Model file for the job. Use its own axes, mm. Round coordinates to 2 decimals unless told otherwise and drop trailing zeros. Loops run counter-clockwise (first coordinate to the right, second up) from the corner with the lowest first, then second, coordinate; pieces in that order, holes last.
from build123d import *

# Parameters (mm, degrees)
SKETCH_1_W      = 190
SKETCH_1_H      = 50
SKETCH_1_R      = 4.5
EXTRUDE_1_DEPTH = 7.25


with BuildPart() as part:
    # 草图1 → 凸台-拉伸1 (new, symmetric)
    with BuildSketch(Plane.XY):
        Rectangle(SKETCH_1_W, SKETCH_1_H)
        with Locations(Location((-42, 0, 0), (0, 0, 180))):
            Circle(SKETCH_1_R, mode=Mode.SUBTRACT)
        with Locations(Location((42, 0, 0), (0, 0, 180))):
            Circle(SKETCH_1_R, mode=Mode.SUBTRACT)
    extrude(amount=EXTRUDE_1_DEPTH, both=True)


solid = part.part
Q1. Slice it at B-B on x = 42. Give the cut face in (y, z).
Q2. Slice it at A-A on y = 0. Give the cut face in (x, z).
Q3. Probe line 1 (Y direction, x = -42, z = 4.25); line 2 (X direction, y = 0.5, z = 6); line 3 (X direction, y = -2, z = -6.5). List the from-to ranges inside material, lowest first.
Q4. Pull direction Y, two halves, no side cores. Call faces 1 (the face through (-46.292, -1.352, -0.101)), 2 (the face through (-1, -25, 0)), 3 (the face through (-1, 25, 0)), 4 (the face through (37.708, -1.352, -0.101)): pulls with the +Y half, pulls with the -Y half, needs draft (parallel to the pull), parting line crosses it, or undercut.
Reply:
1. outline: (-25, -7.25) - (-4.5, -7.25) - (-4.5, 7.25) - (-25, 7.25) - close; (4.5, -7.25) - (25, -7.25) - (25, 7.25) - (4.5, 7.25) - close
2. outline: (-95, -7.25) - (-46.5, -7.25) - (-46.5, 7.25) - (-95, 7.25) - close; (-37.5, -7.25) - (37.5, -7.25) - (37.5, 7.25) - (-37.5, 7.25) - close; (46.5, -7.25) - (95, -7.25) - (95, 7.25) - (46.5, 7.25) - close
3. line 1: y = -25 to -4.5, 4.5 to 25
3. line 2: x = -95 to -46.47, -37.53 to 37.53, 46.47 to 95
3. line 3: x = -95 to -46.03, -37.97 to 37.97, 46.03 to 95
4. face 1: undercut
4. face 2: pulls with the -Y half
4. face 3: pulls with the +Y half
4. face 4: undercut
